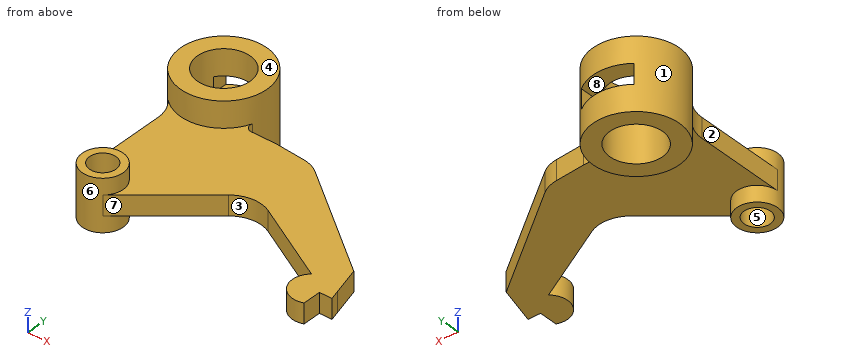
from build123d import *

# Parameters (mm, degrees)
HUB_SKETCH_R        = 19.65
HUB_39_3_DEPTH      = 16.2
LEVER_ARM_DEPTH     = 4.5
PIN_BOSS_DEPTH      = 7.2
PIN_BOSS_DEPTH_BACK = 16.2
PIN_BOSS_SKETCH_R   = 9.3
PIN_HOLE_SKETCH_R   = 6
PIN_HOLE_DEPTH      = 40.2
HUB_BORE_SKETCH_R   = 12
HUB_BORE_DEPTH      = 40.2
HUB_SLOT_DEPTH      = 13.2


with BuildPart() as part:
    # Hub Sketch → Hub Ø39.3 (new, symmetric)
    with BuildSketch(Plane.XY):
        Circle(HUB_SKETCH_R)
    extrude(amount=HUB_39_3_DEPTH, both=True)

    # Lever Arm Sketch → Lever Arm (add, symmetric)
    with BuildSketch(Plane.XY):
        with BuildLine():
            Line((-9.3, -24.700860309), (-9.3, -66))
            ThreePointArc((-9.3, -66), (-3.930349834, -74.428662419), (5.97792477, -73.124213321))
            Line((5.97792477, -73.124213321), (39.595019689, -44.916121374))
            ThreePointArc((39.595019689, -44.916121374), (47.737857787, -41.481873588), (56.401006262, -43.228220821))
            Line((56.401006262, -43.228220821), (92.511102657, -62.858500278))
            ThreePointArc((92.511102657, -62.858500278), (90.79997011, -74.302591391), (101.773667668, -77.973171442))
            Line((101.773667668, -77.973171442), (101.773667668, -69.6))
            Line((101.773667668, -69.6), (107.473667668, -69.6))
            Line((107.473667668, -69.6), (106.267896302, -65.1))
            Line((106.267896302, -65.1), (102.772365267, -52.054500578))
            Line((102.772365267, -52.054500578), (53.950427648, -14.698104885))
            ThreePointArc((53.950427648, -14.698104885), (50.262300823, -12.627051677), (46.142629433, -11.667964344))
            Line((46.142629433, -11.667964344), (32.79273589, -10.5))
            Line((32.79273589, -10.5), (21.372236663, -10.5))
            ThreePointArc((21.372236663, -10.5), (18.924775484, -9.234916071), (18.541476841, -6.506622517))
            ThreePointArc((18.541476841, -6.506622517), (4.442271, -19.141283352), (-13.780519481, -14.007847188))
            ThreePointArc((-13.780519481, -14.007847188), (-10.465401925, -18.903973549), (-9.3, -24.700860309))
        make_face()
    extrude(amount=LEVER_ARM_DEPTH, both=True)

    # Pin Boss Sketch → Pin Boss (add, two sides: drawn at the far end of the back side and taken through both)
    with BuildSketch(Plane.XY.offset(4.5).offset(-PIN_BOSS_DEPTH_BACK)):
        with Locations((0, -66)):
            Circle(PIN_BOSS_SKETCH_R)
    extrude(amount=PIN_BOSS_DEPTH + PIN_BOSS_DEPTH_BACK)

    # Pin Hole Sketch → Pin Hole (cut)
    with BuildSketch(Plane.XY.offset(11.7)):
        with Locations((0, -66)):
            Circle(PIN_HOLE_SKETCH_R)
    extrude(amount=-PIN_HOLE_DEPTH, mode=Mode.SUBTRACT)

    # Hub Bore Sketch → Hub Bore (cut)
    with BuildSketch(Plane.XY.offset(16.2)):
        Circle(HUB_BORE_SKETCH_R)
    extrude(amount=-HUB_BORE_DEPTH, mode=Mode.SUBTRACT)

    # Hub Slot Sketch → Hub Slot (cut)
    with BuildSketch(Plane(origin=(0, 19.65, 0), x_dir=(1, 0, 0), z_dir=(0, 1, 0))):
        Polygon((-12, 0), (-12, 4.5), (12, 4.5), (12, -4.5), (-12, -4.5), align=None)
    extrude(amount=-HUB_SLOT_DEPTH, mode=Mode.SUBTRACT)


solid = part.part
Work out the finished part from the listing and answer in its coordinate system (mm). Face numbers are marked on the shaded views. A direction names the side the tool comes from. Round coordinates to 2 decimals unless told otherwise and drop trailing zeros. Write each loop counter-clockwise with the first axis right and the second up, starting at its lowest first coordinate (ties: lowest second). Pieces come first, ordered by that corner, then holes. Notation, with made-up numbers: (-15, -34) -> (13, -34) arc R7 ccw to (13, -26) -> close; hole circle Ø9 at (39.25, 36). An arc over 180 degrees is marked (long way). Write each question's results on one line, items separated by ' | '.
Item 1: A cutting plane is placed at C-C, the plane z = 13.5. Determine the outline of the cut face in (x, y), plus the area to 3 significant figures.
Result set:
outline: circle Ø39.3 at (0, 0); hole circle Ø24 at (0, 0) | area: 761 mm^2
Item 2: Flat-ended cylindrical pins translate along their axes: P1, Ø10, axis at y = 9.5, z = 0, coming from the -X side; P2, Ø8, axis at x = -2, z = 2, coming from the +Y side; P3, Ø12, axis at y = -6, z = -12.5, coming from the +X side; P4, Ø1.5, axis at x = 11, z = 1, coming from the +Y side. Find the tip coordinate at first contact, or state that the pin passes through.
Result set:
P1: x = -19.13 | P2: y = 19.65 | P3: x = 19.65 | P4: y = 6.45
Item 3: A cutting plane is placed at B-B, the plane y = 0. Determine the outline of the cut face in (x, z), plus the area to 3 significant figures.
Result set:
outline: (-19.65, -16.2) -> (-12, -16.2) -> (-12, 16.2) -> (-19.65, 16.2) -> close; (12, -16.2) -> (19.65, -16.2) -> (19.65, 16.2) -> (12, 16.2) -> close | area: 496 mm^2
Item 4: The mould has two halves that part along X. Classify the marked faces 1, 2, 3 and 4: +X half, -X half, draft (parallel to the pull), parting line (faces both ways), or undercut.
Result set:
face 1: parting line | face 2: -X half | face 3: undercut | face 4: draft
Item 5: A cutting plane is placed at D-D, the plane y = -53.5. Determine the outline of the cut face in (x, z), plus the area to 3 significant figures.
Result set:
outline: (-9.3, -4.5) -> (29.37, -4.5) -> (29.37, 4.5) -> (-9.3, 4.5) -> close; (75.3, -4.5) -> (103.16, -4.5) -> (103.16, 4.5) -> (75.3, 4.5) -> close | area: 599 mm^2
Item 6: A cutting plane is placed at A-A, the plane x = 0. Determine the outline of the cut face in (y, z).
Result set:
outline: (-75.3, -11.7) -> (-72, -11.7) -> (-72, 11.7) -> (-75.3, 11.7) -> close; (-60, -11.7) -> (-56.7, -11.7) -> (-56.7, -4.5) -> (-19.65, -4.5) -> (-19.65, -16.2) -> (-12, -16.2) -> (-12, 16.2) -> (-19.65, 16.2) -> (-19.65, 4.5) -> (-56.7, 4.5) -> (-56.7, 11.7) -> (-60, 11.7) -> close; (12, -16.2) -> (19.65, -16.2) -> (19.65, -4.5) -> (12, -4.5) -> close; (12, 4.5) -> (19.65, 4.5) -> (19.65, 16.2) -> (12, 16.2) -> close
Item 7: Find the intervals of material crossed by line 1 along Y through (x, z) = (0, 6); line 2 along Y through (x, z) = (0, 2.5); line 3 along Y through (x, z) = (1, 11.5), in increasing order. Write a range as [from, to].
Result set:
line 1: [-75.3, -72], [-60, -56.7], [-19.65, -12], [12, 19.65] | line 2: [-75.3, -72], [-60, -12] | line 3: [-75.25, -71.92], [-60.08, -56.75], [-19.62, -11.96], [11.96, 19.62]
Item 8: Which of the six approach directions +Z, -Z, +X, -X, +Y, -Y give full straight-line access (tool end or side, diameter ignored) to the marked faces 5, 6, 7 and 8?
Result set:
face 5: +Z, -Z | face 6: none | face 7: +Z, -Z, -Y | face 8: +Y
